```python
from build123d import *

# Parameters (mm, degrees)
SKETCH_1_R      = 5
EXTRUDE_1_DEPTH = 2.5


with BuildPart() as part:
    # 草图1 → 凸台-拉伸1 (new, symmetric)
    with BuildSketch(Plane.XY):
        with BuildLine():
            Line((8, 0), (8, 18))
            ThreePointArc((8, 18), (0, 26), (-8, 18))
            Line((-8, 18), (-8, 0))
            Line((-8, 0), (8, 0))
        make_face()
        with Locations((0, 18)):
            Circle(SKETCH_1_R, mode=Mode.SUBTRACT)
    extrude(amount=EXTRUDE_1_DEPTH, both=True)


solid = part.part
```
Could you check a few things on this model? Use its own coordinates, in mm. Coordinates: 2 decimals unless noted, no trailing zeros. Write each loop counter-clockwise with the first axis right and the second up, starting at its lowest first coordinate (ties: lowest second). Pieces come first, ordered by that corner, then holes. Notation, with made-up numbers: (52, 84.25) -> (80, 84.25) arc R15 cw to (80, 106.25) -> close; hole circle Ø1 at (-18, -17.5). An arc over 180 degrees is marked (long way). One line per question, with ' | ' between items. Start each with the question number.
1. If we section it at B-B (z = 0.9): Please give me the cut outline in (x, y), and give its area (3 significant figures).
2. Thinking about a two-plate mould opening in Y: for faces 1 (the face through (0, 26, 0)), 2 (the face through (0, 0, 0)), 3 (the face through (-1.08, 13.12, -0.04)), 4 (the face through (-8, 9, 0)), which applies, pulls with the +Y half, pulls with the -Y half, needs draft (parallel to the pull), parting line crosses it, or undercut?
3. Please list where these lines run through material, in increasing order: line 1 along Y through (x, z) = (0, -1.05); line 2 along Y through (x, z) = (1, -1.55); line 3 along X through (y, z) = (16.5, 2.1).
4. If we section it at A-A (x = 0): Please give me the cut outline in (y, z), and give its area (3 significant figures).
5. If we section it at C-C (x = 4.5): Please give me the cut outline in (y, z), and give its area (3 significant figures).
6. Will this pin go through, and if not, where does the flat tip stop? P1, Ø9, axis at x = 0, y = 18, coming from the +Z side.
Return value:
1) outline: (-8, 0) -> (8, 0) -> (8, 18) arc R8 ccw to (-8, 18) -> close; hole circle Ø10 at (0, 18) | area: 310 mm²
2) face 1: pulls with the +Y half | face 2: pulls with the -Y half | face 3: undercut | face 4: needs draft
3) line 1: y = 0 to 13, 23 to 26 | line 2: y = 0 to 13.1, 22.9 to 25.94 | line 3: x = -8 to -4.77, 4.77 to 8
4) outline: (0, -2.5) -> (13, -2.5) -> (13, 2.5) -> (0, 2.5) -> close; (23, -2.5) -> (26, -2.5) -> (26, 2.5) -> (23, 2.5) -> close | area: 80.0 mm²
5) outline: (0, -2.5) -> (15.82, -2.5) -> (15.82, 2.5) -> (0, 2.5) -> close; (20.18, -2.5) -> (24.61, -2.5) -> (24.61, 2.5) -> (20.18, 2.5) -> close | area: 101 mm²
6) P1: passes through
